Model file for the job. Use its own axes, mm. Round coordinates to 2 decimals unless told otherwise and drop trailing zeros. Order: outer loops, then holes, each group sorted by start corner. A loop starts at its lowest first (then second) coordinate and runs counter-clockwise, first axis right, second up. Notation, with made-up numbers: (-11.5, 33.5) - (47.5, 33.5) arc R30 ccw to (47.5, 72.5) - close; hole circle Ø6 at (71, 1). An arc over 180 degrees is marked (long way). Write item = value, one per line.
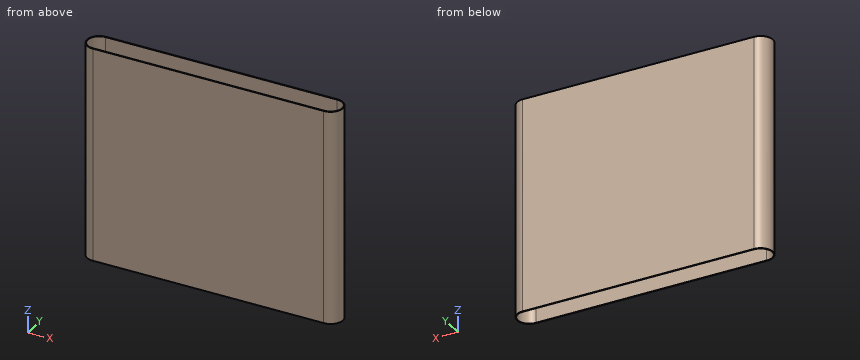
```python
from build123d import *

# Parameters (mm, degrees)
EXTRUDE_1_DEPTH      = 350
EXTRUDE_2_DEPTH      = 352
EXTRUDE_2_DEPTH_BACK = 361


with BuildPart() as part:
    # 草图1 → 拉伸-薄壁1 (new, symmetric)
    with BuildSketch(Plane.XY):
        with BuildLine():
            Line((381.234257801, -39.979968693), (-381.234257801, -39.979968693))
            ThreePointArc((-381.234257801, -39.979968693), (-422.49499186, -0.632950347), (-382.5, 40))
            Line((-382.5, 40), (382.5, 40))
            ThreePointArc((382.5, 40), (422.49499186, -0.632950347), (381.234257801, -39.979968693))
        make_face()
        with BuildLine():
            Line((381.26631524, -37.979968693), (-381.26631524, -37.979968693))
            ThreePointArc((-381.26631524, -37.979968693), (-420.494991843, -0.616923686), (-382.5, 38))
            Line((-382.5, 38), (382.5, 38))
            ThreePointArc((382.5, 38), (420.494991843, -0.616923686), (381.26631524, -37.979968693))
        make_face(mode=Mode.SUBTRACT)
    extrude(amount=EXTRUDE_1_DEPTH, both=True)

    # 草图4 → 凸台-拉伸2 (add, two sides: drawn at the far end of the back side and taken through both)
    with BuildSketch(Plane(origin=(0, 0, 0), x_dir=(0, 0, -1), z_dir=(1, 0, 0)).offset(-EXTRUDE_2_DEPTH_BACK)):
        Polygon((4, 38), (-4, 38), (-2.5, 33), (2.5, 33), align=None)
    extrude(amount=EXTRUDE_2_DEPTH + EXTRUDE_2_DEPTH_BACK)


solid = part.part
```
1) Wall check: line 1 along Y through (x, z) = (-28, -256); line 2 along X through (y, z) = (-1.5, 224); line 3 along X through (y, z) = (-16, -204.5). Give the ranges that are in metal, low to high.
Conclusion:
line_1 = -39.98 to -37.98, 38 to 40
line_2 = -422.47 to -420.47, 420.47 to 422.47
line_3 = -419.16 to -416.97, 416.97 to 419.16
2) Cut at C-C (x = 88). Write the cut outline in (y, z).
Conclusion:
outline = (-39.98, -350) - (-37.98, -350) - (-37.98, 350) - (-39.98, 350) - close; (33, -2.5) - (38, -4) - (38, -350) - (40, -350) - (40, 350) - (38, 350) - (38, 4) - (33, 2.5) - close
3) Cut at A-A (y = 0). Write the cut outline in (x, z).
Conclusion:
outline = (-422.5, -350) - (-420.5, -350) - (-420.5, 350) - (-422.5, 350) - close; (420.5, -350) - (422.5, -350) - (422.5, 350) - (420.5, 350) - close
4) Flat gauge pins, fed straight in: pin 1 Ø1.5 at (x, z) = (117.5, 0) entering from -Y; pin 2 Ø10 at (y, z) = (9, 247.5) entering from -X; pin 3 Ø2.5 at (y, z) = (35.5, -1.5) entering from +X. Where does each tip first touch, or does it go through?
Conclusion:
pin_1 = -39.98
pin_2 = -422.3
pin_3 = 403.16
5) Cut at B-B (z = -222.5). Write the cut outline in (x, y).
Conclusion:
outline = (-382.5, 40) arc R40 ccw (long way) to (-381.23, -39.98) - (381.23, -39.98) arc R40 ccw (long way) to (382.5, 40) - close; hole (-382.5, 38) arc R38 ccw (long way) to (-381.27, -37.98) - (381.27, -37.98) arc R38 ccw (long way) to (382.5, 38) - close
